Read the model definition and answer for the solid it produces. Units are mm, in the model's axes. Coordinates: 2 decimals unless noted, no trailing zeros. Loops run counter-clockwise (first coordinate to the right, second up) from the corner with the lowest first, then second, coordinate; pieces in that order, holes last. Notation, with made-up numbers: (81, 75) -> (119, 75) arc R18 cw to (119, 103) -> close; hole circle Ø2 at (47, 22.25). An arc over 180 degrees is marked (long way). Answer as a JSON object with one key per item and string values. Group by question number.
1) Determine the mould class of faces 1 (the face through (-52.5, 0, 2)), 2 (the face through (-1, -4, 2)), 3 (the face through (1.216, 1.115, 2.465)), 4 (the face through (-1, 4, 2)) for opening direction Y: released by +Y, released by -Y, zero draft, split by the parting line, or undercut.
2) Section C-C, the plane x = -40 is taken. Give the vertices of the cut face in (y, z), plus the area to 3 significant figures.
3) Section A-A, the plane y = 0 is taken. Give the vertices of the cut face in (x, z), plus the area to 4 significant figures.
4) Section B-B, the plane z = 1.65 is taken. Give the vertices of the cut face in (x, y), plus the area to 3 significant figures.
5) Consider probe 1 along Y at (x, z) = (-40, 2.2); probe 2 along X at (y, z) = (0.5, 0.6); probe 3 along X at (y, z) = (-1.25, 3.9). Determine where each line is inside the solid, lowest interval first. Write a range as [from, to].
from build123d import *

# Parameters (mm, degrees)
SKETCH1_W           = 105
SKETCH1_H           = 8
BOSS_EXTRUDE1_DEPTH = 5
M4_TAPPED_HOLE2_D   = 3.3


with BuildPart() as part:
    # Sketch1 → Boss-Extrude1 (new body)
    with BuildSketch(Plane.XY):
        Rectangle(SKETCH1_W, SKETCH1_H)
    extrude(amount=BOSS_EXTRUDE1_DEPTH)

    # M4 Tapped Hole2 (through all)
    with Locations(Plane.XY.offset(5)):
        with Locations((-40, 0), (0, 0), (40, 0)):
            Hole(M4_TAPPED_HOLE2_D / 2)


solid = part.part
Determined:
{
 "1": {"face 1": "zero draft", "face 2": "released by -Y", "face 3": "undercut", "face 4": "released by +Y"},
 "2": {"outline": "(-4, 0) -> (-1.65, 0) -> (-1.65, 5) -> (-4, 5) -> close; (1.65, 0) -> (4, 0) -> (4, 5) -> (1.65, 5) -> close", "area": "23.5 mm²"},
 "3": {"outline": "(-52.5, 0) -> (-41.65, 0) -> (-41.65, 5) -> (-52.5, 5) -> close; (-38.35, 0) -> (-1.65, 0) -> (-1.65, 5) -> (-38.35, 5) -> close; (1.65, 0) -> (38.35, 0) -> (38.35, 5) -> (1.65, 5) -> close; (41.65, 0) -> (52.5, 0) -> (52.5, 5) -> (41.65, 5) -> close", "area": "475.5 mm²"},
 "4": {"outline": "(-52.5, -4) -> (52.5, -4) -> (52.5, 4) -> (-52.5, 4) -> close; hole circle Ø3.3 at (-40, 0); hole circle Ø3.3 at (0, 0); hole circle Ø3.3 at (40, 0)", "area": "814 mm²"},
 "5": {"probe 1": "[-4, -1.65], [1.65, 4]", "probe 2": "[-52.5, -41.57], [-38.43, -1.57], [1.57, 38.43], [41.57, 52.5]", "probe 3": "[-52.5, -41.08], [-38.92, -1.08], [1.08, 38.92], [41.08, 52.5]"}
}
